Here's how the part is built. I have some questions about the finished solid (model axes, mm). A direction names the side the tool comes from. Coordinates: 2 decimals unless noted, no trailing zeros. Write each loop counter-clockwise with the first axis right and the second up, starting at its lowest first coordinate (ties: lowest second). Pieces come first, ordered by that corner, then holes.
from build123d import *

# Parameters (mm, degrees)
SKETCH_1_W                    = 100
SKETCH_1_H                    = 100
EXTRUDE_1_DEPTH               = 15
HOLE_WIZARD_M10_1_D           = 12
HOLE_WIZARD_M10_1_CBORE_D     = 18
HOLE_WIZARD_M10_1_CBORE_DEPTH = 10.6
CHAMFER_1_SIZE                = 10
SKETCH_11_R                   = 27.5
CUT_EXTRUDE_4_DEPTH           = 13
HOLE_WIZARD_M6_1_D            = 5
HOLE_WIZARD_M6_1_DEPTH        = 15
HOLE_WIZARD_M6_1_TIP          = 1.502151548
SKETCH_14_R                   = 24.5
CUT_EXTRUDE_5_DEPTH           = 72.895757872


with BuildPart() as part:
    # 草图1 → 凸台-拉伸1 (new body)
    with BuildSketch(Plane.XY):
        Rectangle(SKETCH_1_W, SKETCH_1_H)
    extrude(amount=EXTRUDE_1_DEPTH)

    # M10 六角凹头螺钉的柱形沉头孔1 (through all)
    with Locations(Plane(origin=(0, 0, 0), x_dir=(-1, 0, 0), z_dir=(0, 0, -1))):
        with Locations((-32.5, 32.5), (32.5, 32.5), (32.5, -32.5), (-32.5, -32.5)):
            CounterBoreHole(HOLE_WIZARD_M10_1_D / 2, HOLE_WIZARD_M10_1_CBORE_D / 2, HOLE_WIZARD_M10_1_CBORE_DEPTH)

    # 倒角1
    chamfer_1_edges = [part.edges().sort_by_distance(p)[0] for p in [
        (50, -50, 7.5),
        (-50, -50, 7.5),
        (-50, 50, 7.5),
        (50, 50, 7.5),
    ]]
    chamfer(chamfer_1_edges, length=CHAMFER_1_SIZE)

    # 草图11 → 切除-拉伸4 (cut)
    with BuildSketch(Plane(origin=(0, 0, 0), x_dir=(-1, 0, 0), z_dir=(0, 0, -1))):
        Circle(SKETCH_11_R)
    extrude(amount=-CUT_EXTRUDE_4_DEPTH, mode=Mode.SUBTRACT)

    # M6 螺纹孔1
    with Locations(Plane(origin=(0, 0, 0), x_dir=(-1, 0, 0), z_dir=(0, 0, -1))):
        with Locations((0, 31), (31, 0), (0, -31), (-31, 0)):
            Hole(HOLE_WIZARD_M6_1_D / 2, depth=HOLE_WIZARD_M6_1_DEPTH)
            with Locations((0, 0, -(HOLE_WIZARD_M6_1_DEPTH + HOLE_WIZARD_M6_1_TIP / 2))):  # 118° drill point
                Cone(0, HOLE_WIZARD_M6_1_D / 2, HOLE_WIZARD_M6_1_TIP, mode=Mode.SUBTRACT)

    # 草图14 → 切除-拉伸5 (cut, through all)
    with BuildSketch(Plane(origin=(0, 0, 13), x_dir=(-1, 0, 0), z_dir=(0, 0, -1))):
        Circle(SKETCH_14_R)
    extrude(amount=-CUT_EXTRUDE_5_DEPTH, mode=Mode.SUBTRACT)


solid = part.part
1. I want a section at A-A (z = 3.25). State how many separate pieces and enclosed holes the cut face has, then the cut area to 3 significant figures.
2. I want a section at B-B (y = 0). List the corners of the cut face in (x, z) for me.
3. On a 3-axis mill with a long thin cutter (end or side, diameter ignored), from which of +Z, -Z, +X, -X, +Y, -Y can I reach the whole of each face in a straight line? I mean faces 4 (the face through (-31.328, 41.423, 5.226)), 5 (the face through (-12, 23, 15)). Say none if no direction works.
4. For pin 1 Ø9.5 at (x, y) = (32.5, 32.5) entering from -Z; pin 2 Ø14 at (x, y) = (32.5, -32.5) entering from -Z, each with a flat end and sliding along its axis, tell me the tip position at first contact or that it passes through.
5. Thinking about a two-plate mould opening in Y: for faces 1 (the face through (-45, -45, 7)), 2 (the face through (22, -22, 0)), 3 (the face through (-38.4, -34.4, 10.6)), which applies, pulls with the +Y half, pulls with the -Y half, needs draft (parallel to the pull), parting line crosses it, or undercut?
6. If I drill on line 1 (Y direction, x = 0, z = 11.5); line 2 (Y direction, x = 32.5, z = 7); line 3 (X direction, y = -29, z = 8), over which ranges is the centre line in solid material (lowest first)?
7. I want a section at D-D (y = 35.5). List the corners of the cut face in (x, z) for me, then the cut area to 3 significant figures.
Response values:
1. separate pieces: 1
1. enclosed holes: 9
1. area: 6,330 mm2
2. outline: (-50, 0) - (-33.5, 0) - (-33.5, 15) - (-50, 15) - close; (-28.5, 0) - (-27.5, 0) - (-27.5, 13) - (-24.5, 13) - (-24.5, 15) - (-28.5, 15) - close; (24.5, 13) - (27.5, 13) - (27.5, 0) - (28.5, 0) - (28.5, 15) - (24.5, 15) - close; (33.5, 0) - (50, 0) - (50, 15) - (33.5, 15) - close
3. face 4: -Z
3. face 5: +Z, +X, -X, +Y, -Y
4. pin 1: passes through
4. pin 2: stops at z = 10.6
5. face 1: pulls with the -Y half
5. face 2: needs draft
5. face 3: undercut
6. line 1: y = -50 to -33.5, -28.5 to -27.5, 27.5 to 28.5, 33.5 to 50
6. line 2: y = -50 to -41.5, -23.5 to -2, 2 to 23.5, 41.5 to 50
6. line 3: x = -50 to -40.79, -24.21 to -1.5, 1.5 to 24.21, 40.79 to 50
7. outline: (-50, 0) - (-40.99, 0) - (-40.99, 10.6) - (-37.7, 10.6) - (-37.7, 15) - (-50, 15) - close; (-27.3, 10.6) - (-24.01, 10.6) - (-24.01, 0) - (24.01, 0) - (24.01, 10.6) - (27.3, 10.6) - (27.3, 15) - (-27.3, 15) - close; (37.7, 10.6) - (40.99, 10.6) - (40.99, 0) - (50, 0) - (50, 15) - (37.7, 15) - close
7. area: 1,050 mm2
